from build123d import *

# Parameters (mm, degrees)
SKETCH_1_R               = 13.5
SKETCH_1_R_2             = 8.5
EXTRUDE_1_DEPTH          = 25
SKETCH_2_W               = 1.5
SKETCH_2_H               = 2
PATTERN_LINEAR_1_COUNT   = 6
PATTERN_LINEAR_1_PITCH   = 3
MIRROR_1_COPY_1_SKETCH_W = 1.5
MIRROR_1_COPY_1_SKETCH_H = 2
MIRROR_1_COPY_2_SKETCH_W = 1.5
MIRROR_1_COPY_2_SKETCH_H = 2
MIRROR_1_COPY_3_SKETCH_W = 1.5
MIRROR_1_COPY_3_SKETCH_H = 2
MIRROR_1_COPY_4_SKETCH_W = 1.5
MIRROR_1_COPY_4_SKETCH_H = 2
MIRROR_1_COPY_5_SKETCH_W = 1.5
MIRROR_1_COPY_5_SKETCH_H = 2
MIRROR_1_COPY_6_SKETCH_W = 1.5
MIRROR_1_COPY_6_SKETCH_H = 2
SKETCH_3_R               = 10.5
CUT_EXTRUDE_1_DEPTH      = 5


with BuildPart() as part:
    # 草图1 → 凸台-拉伸1 (new, symmetric)
    with BuildSketch(Plane.XY):
        Circle(SKETCH_1_R)
        Circle(SKETCH_1_R_2, mode=Mode.SUBTRACT)
    extrude(amount=EXTRUDE_1_DEPTH, both=True)

    # 草图2 → 切除-旋转1 (revolve, cut)
    with BuildSketch(Plane(origin=(0, 0, 0), x_dir=(1, 0, 0), z_dir=(0, 1, 0))):
        with Locations((12.75, 0)):
            Rectangle(SKETCH_2_W, SKETCH_2_H)
    cut_revolve_1 = revolve(axis=Axis((0, 0, 0), (0, 0, -1)), mode=Mode.SUBTRACT)

    # 阵列(线性)1: 切除-旋转1 ×6
    with Locations(*[(0, 0, -i * PATTERN_LINEAR_1_PITCH) for i in range(1, PATTERN_LINEAR_1_COUNT)]):
        add(cut_revolve_1, mode=Mode.SUBTRACT)

    # 镜向1 copy 1 sketch → 镜向1 copy 1 (revolve, cut)
    with BuildSketch(Plane(origin=(0, 0, 3), x_dir=(1, 0, 0), z_dir=(0, 1, 0))):
        with Locations((12.75, 0)):
            Rectangle(MIRROR_1_COPY_1_SKETCH_W, MIRROR_1_COPY_1_SKETCH_H)
    revolve(axis=Axis((0, 0, 3), (0, 0, -1)), mode=Mode.SUBTRACT)

    # 镜向1 copy 2 sketch → 镜向1 copy 2 (revolve, cut)
    with BuildSketch(Plane(origin=(0, 0, 6), x_dir=(1, 0, 0), z_dir=(0, 1, 0))):
        with Locations((12.75, 0)):
            Rectangle(MIRROR_1_COPY_2_SKETCH_W, MIRROR_1_COPY_2_SKETCH_H)
    revolve(axis=Axis((0, 0, 6), (0, 0, -1)), mode=Mode.SUBTRACT)

    # 镜向1 copy 3 sketch → 镜向1 copy 3 (revolve, cut)
    with BuildSketch(Plane(origin=(0, 0, 9), x_dir=(1, 0, 0), z_dir=(0, 1, 0))):
        with Locations((12.75, 0)):
            Rectangle(MIRROR_1_COPY_3_SKETCH_W, MIRROR_1_COPY_3_SKETCH_H)
    revolve(axis=Axis((0, 0, 9), (0, 0, -1)), mode=Mode.SUBTRACT)

    # 镜向1 copy 4 sketch → 镜向1 copy 4 (revolve, cut)
    with BuildSketch(Plane(origin=(0, 0, 12), x_dir=(1, 0, 0), z_dir=(0, 1, 0))):
        with Locations((12.75, 0)):
            Rectangle(MIRROR_1_COPY_4_SKETCH_W, MIRROR_1_COPY_4_SKETCH_H)
    revolve(axis=Axis((0, 0, 12), (0, 0, -1)), mode=Mode.SUBTRACT)

    # 镜向1 copy 5 sketch → 镜向1 copy 5 (revolve, cut)
    with BuildSketch(Plane(origin=(0, 0, 15), x_dir=(1, 0, 0), z_dir=(0, 1, 0))):
        with Locations((12.75, 0)):
            Rectangle(MIRROR_1_COPY_5_SKETCH_W, MIRROR_1_COPY_5_SKETCH_H)
    revolve(axis=Axis((0, 0, 15), (0, 0, -1)), mode=Mode.SUBTRACT)

    # 镜向1 copy 6 sketch → 镜向1 copy 6 (revolve, cut)
    with BuildSketch(Plane(origin=(0, 0, 0), x_dir=(1, 0, 0), z_dir=(0, 1, 0))):
        with Locations((12.75, 0)):
            Rectangle(MIRROR_1_COPY_6_SKETCH_W, MIRROR_1_COPY_6_SKETCH_H)
    revolve(axis=Axis((0, 0, 0), (0, 0, -1)), mode=Mode.SUBTRACT)

    # 草图3 → 切除-拉伸1 (cut)
    with BuildSketch(Plane.XY.offset(25)):
        Circle(SKETCH_3_R)
    cut_extrude_1 = extrude(amount=-CUT_EXTRUDE_1_DEPTH, mode=Mode.SUBTRACT)

    # 镜向2: 切除-拉伸1 across plane
    add(cut_extrude_1.mirror(Plane.XY), mode=Mode.SUBTRACT)


solid = part.part
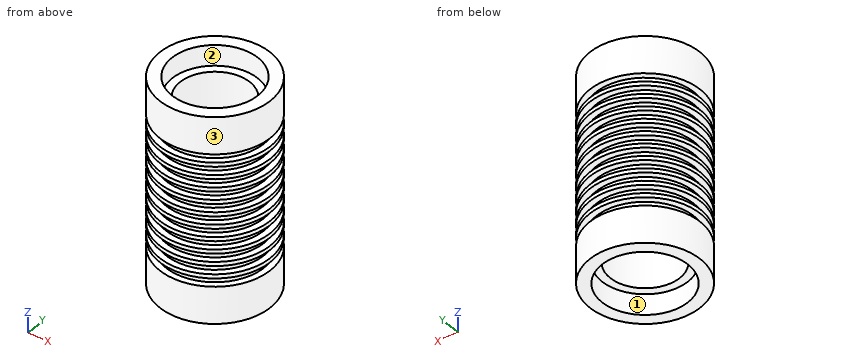
The model under review builds one solid part; all positions refer to its coordinate system, in mm. Face numbers are marked on the shaded views. Round coordinates to 2 decimals unless told otherwise and drop trailing zeros. Use a Markdown table: item, result. Add a question column.
Q1. The part is to be moulded in two halves that separate along Y. For the marked faces 1, 2 and 3, say which applies: pulls with the +Y half, pulls with the -Y half, needs draft (parallel to the pull), parting line crosses it, or undercut.
Q2. To check wall thickness, follow line 1 (Y direction, x = 0, z = -3.5); line 2 (Z direction, x = 7.75, y = 6). State the ranges of each line that lie inside material, in increasing order.
Q3. Insertion check: pin 1 (12 mm diameter, centred on y = 10, z = 7.5, fed in from +X); pin 2 (6 mm diameter, centred on y = -9.5, z = 12, fed in from +X); pin 3 (1 mm diameter, centred on y = 4.5, z = 17.5, fed in from -X); pin 4 (15.5 mm diameter, centred on x = 0, y = 0, fed in from -Z). Each pin has a flat end and moves straight along its axis. Give the tip position at first contact, or say it passes through.
Findings below:
| question | item | result |
|---|---|---|
| 1 | face 1 | undercut |
| 1 | face 2 | undercut |
| 1 | face 3 | parting line crosses it |
| 2 | line 1 | y = -12 to -8.5, 8.5 to 12 |
| 2 | line 2 | z = -20 to 20 |
| 3 | pin 1 | stops at x = 12.89 |
| 3 | pin 2 | stops at x = 11.74 |
| 3 | pin 3 | stops at x = -12.89 |
| 3 | pin 4 | passes through |
